from build123d import *

# Parameters (mm, degrees)
SKETCH1_R           = 0.55
THIGH1_LENGTH_DEPTH = 0.5


with BuildPart() as part:
    # Sketch1 → Thigh1 length (new, symmetric)
    with BuildSketch(Plane.XY):
        with BuildLine():
            Line((-10.75, 1), (10.75, 1))
            ThreePointArc((10.75, 1), (11.75, 0), (10.75, -1))
            Line((10.75, -1), (-10.75, -1))
            ThreePointArc((-10.75, -1), (-11.75, 0), (-10.75, 1))
        make_face()
        with Locations((-10.75, 0)):
            Circle(SKETCH1_R, mode=Mode.SUBTRACT)
        with Locations((10.75, 0)):
            Circle(SKETCH1_R, mode=Mode.SUBTRACT)
        with Locations((-6.75, 0)):
            Circle(SKETCH1_R, mode=Mode.SUBTRACT)
        with Locations((7.75, 0)):
            Circle(SKETCH1_R, mode=Mode.SUBTRACT)
    extrude(amount=THIGH1_LENGTH_DEPTH, both=True)


solid = part.part
Build history of the part. All positions in model axes, mm. Give positions to 0.01 mm unless a question says otherwise; leave off trailing zeros. Loops run counter-clockwise (first coordinate to the right, second up) from the corner with the lowest first, then second, coordinate; pieces in that order, holes last. Notation, with made-up numbers: (8, 30.25) - (64, 30.25) arc R18 cw to (64, 38.25) - close; hole circle Ø6 at (82.25, -3). An arc over 180 degrees is marked (long way). Write item = value, one per line. Start each with the question number.
1) Band-saw the part on B-B on z = -0.2. Give the cut face in (x, y), plus the area to 3 significant figures.
2) Band-saw the part on A-A on x = -6.75. Give the cut face in (y, z), plus the area to 3 significant figures.
3) Probe probe 1 along X at (y, z) = (0.05, 0.4); probe 2 along Y at (x, z) = (10.75, 0.25); probe 3 along X at (y, z) = (-0.4, 0.45). List the from-to ranges inside material, lowest first. Write a range as from..to.
4) Pull direction X, two halves, no side cores. Call faces 1 (the cylindrical face through (-11.3, 0, 0)), 2 (the cylindrical face through (11.75, 0.02, 0.01)), 3 (the cylindrical face through (-7.3, 0, 0)), 4 (the flat face through (0, 0, -0.5)): +X half, -X half, draft (parallel to the pull), parting line (faces both ways), or undercut.
5) Band-saw the part on C-C on y = 0. Give the cut face in (x, z), plus the area to 3 significant figures.
Final values:
q1.outline = (-10.75, -1) - (10.75, -1) arc R1 ccw to (10.75, 1) - (-10.75, 1) arc R1 ccw to start; hole circle Ø1.1 at (-10.75, 0); hole circle Ø1.1 at (-6.75, 0); hole circle Ø1.1 at (7.75, 0); hole circle Ø1.1 at (10.75, 0)
q1.area = 42.3 mm²
q2.outline = (-1, -0.5) - (-0.55, -0.5) - (-0.55, 0.5) - (-1, 0.5) - close; (0.55, -0.5) - (1, -0.5) - (1, 0.5) - (0.55, 0.5) - close
q2.area = 0.900 mm²
q3.probe_1 = -11.75..-11.3, -10.2..-7.3, -6.2..7.2, 8.3..10.2, 11.3..11.75
q3.probe_2 = -1..-0.55, 0.55..1
q3.probe_3 = -11.67..-11.13, -10.37..-7.13, -6.37..7.37, 8.13..10.37, 11.13..11.67
q4.face_1 = undercut
q4.face_2 = +X half
q4.face_3 = undercut
q4.face_4 = draft
q5.outline = (-11.75, -0.5) - (-11.3, -0.5) - (-11.3, 0.5) - (-11.75, 0.5) - close; (-10.2, -0.5) - (-7.3, -0.5) - (-7.3, 0.5) - (-10.2, 0.5) - close; (-6.2, -0.5) - (7.2, -0.5) - (7.2, 0.5) - (-6.2, 0.5) - close; (8.3, -0.5) - (10.2, -0.5) - (10.2, 0.5) - (8.3, 0.5) - close; (11.3, -0.5) - (11.75, -0.5) - (11.75, 0.5) - (11.3, 0.5) - close
q5.area = 19.1 mm²
